The figure shows three views and two pictorial views of one solid part (mm, origin at its lowest corner). Answer the questions. Give positions to 0.01 mm unless a question says otherwise; leave off trailing zeros. Write each loop counter-clockwise with the first axis right and the second up, starting at its lowest first coordinate (ties: lowest second). Pieces come first, ordered by that corner, then holes. Notation, with made-up numbers: M -0.5,-17.75 L 40.5,-17.75 A24 cw 40.5,12.25 Z; hole C -16,-13 d6. An arc over 180 degrees is marked long. Return JSON: item names as keys, results as strings.
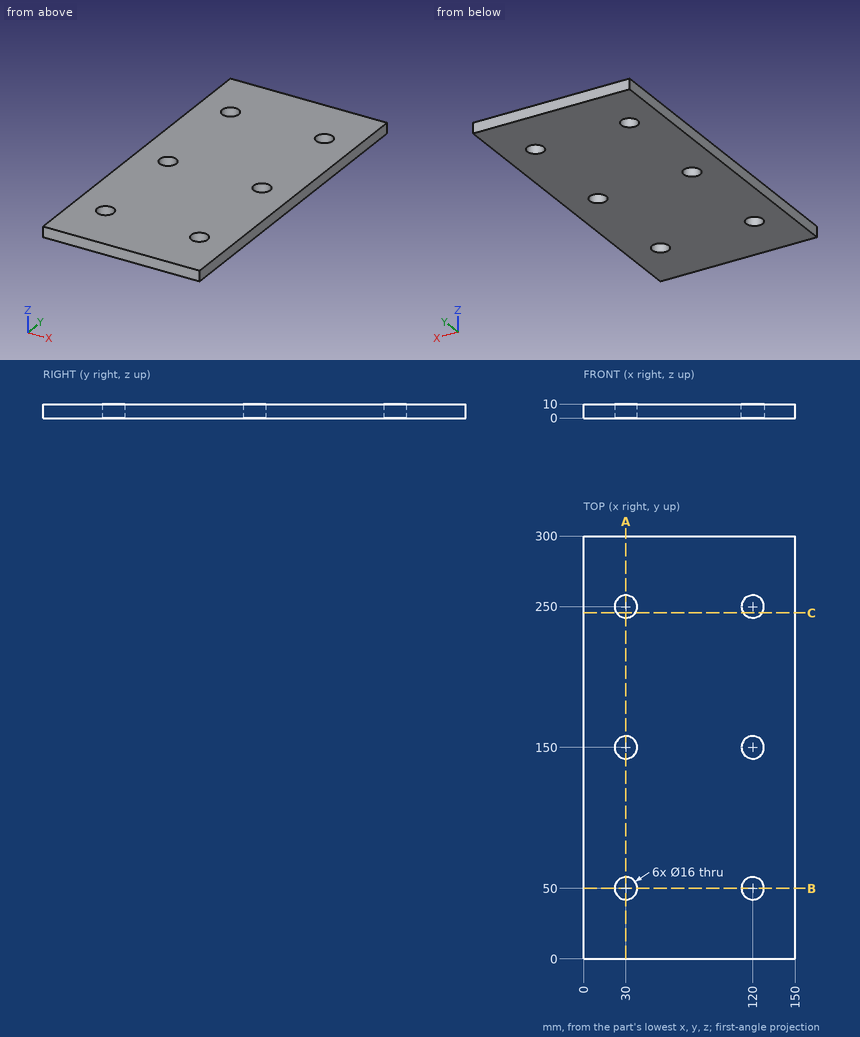
Item 1: Find the intervals of material crossed by line 1 (Y direction, x = 120, z = 7.5); line 2 (Y direction, x = 115.5, z = 8.75); line 3 (X direction, y = 243, z = 2.5), in increasing order.
Geometry results:
{"line 1": "y = 0 to 42, 58 to 142, 158 to 242, 258 to 300", "line 2": "y = 0 to 43.39, 56.61 to 143.39, 156.61 to 243.39, 256.61 to 300", "line 3": "x = 0 to 26.13, 33.87 to 116.13, 123.87 to 150"}
Item 2: A cutting plane is placed at A-A, the plane x = 30. Write down the section's boundary in (y, z).
Geometry results:
{"outline": "M 0,0 L 42,0 L 42,10 L 0,10 Z; M 58,0 L 142,0 L 142,10 L 58,10 Z; M 158,0 L 242,0 L 242,10 L 158,10 Z; M 258,0 L 300,0 L 300,10 L 258,10 Z"}
Item 3: Given pin 1 Ø9.5 at (x, y) = (120, 50) entering from +Z, flat-ended and moving along its own axis, determine where the tip first touches the part or whether it passes through.
Geometry results:
{"pin 1": "passes through"}
Item 4: A cutting plane is placed at B-B, the plane y = 50. Write down the section's boundary in (x, z), plus the area to 3 significant figures.
Geometry results:
{"outline": "M 0,0 L 22,0 L 22,10 L 0,10 Z; M 38,0 L 112,0 L 112,10 L 38,10 Z; M 128,0 L 150,0 L 150,10 L 128,10 Z", "area": "1,180 mm2"}
Item 5: A cutting plane is placed at C-C, the plane y = 245.5. Write down the section's boundary in (x, z), plus the area to 3 significant figures.
Geometry results:
{"outline": "M 0,0 L 23.39,0 L 23.39,10 L 0,10 Z; M 36.61,0 L 113.39,0 L 113.39,10 L 36.61,10 Z; M 126.61,0 L 150,0 L 150,10 L 126.61,10 Z", "area": "1,240 mm2"}
